Verification items for this drawing (mm, ordinates from the low corner). Coordinates: 2 decimals unless noted, no trailing zeros. Order: outer loops, then holes, each group sorted by start corner. A loop starts at its lowest first (then second) coordinate and runs counter-clockwise, first axis right, second up. Notation, with made-up numbers: (-27, -35.5) -> (-7, -35.5) arc R11 ccw to (-7, -21.5) -> close; hole circle Ø8 at (85, 39.5). An arc over 180 degrees is marked (long way). Answer in a Markdown table with one row per item. Add a question column.
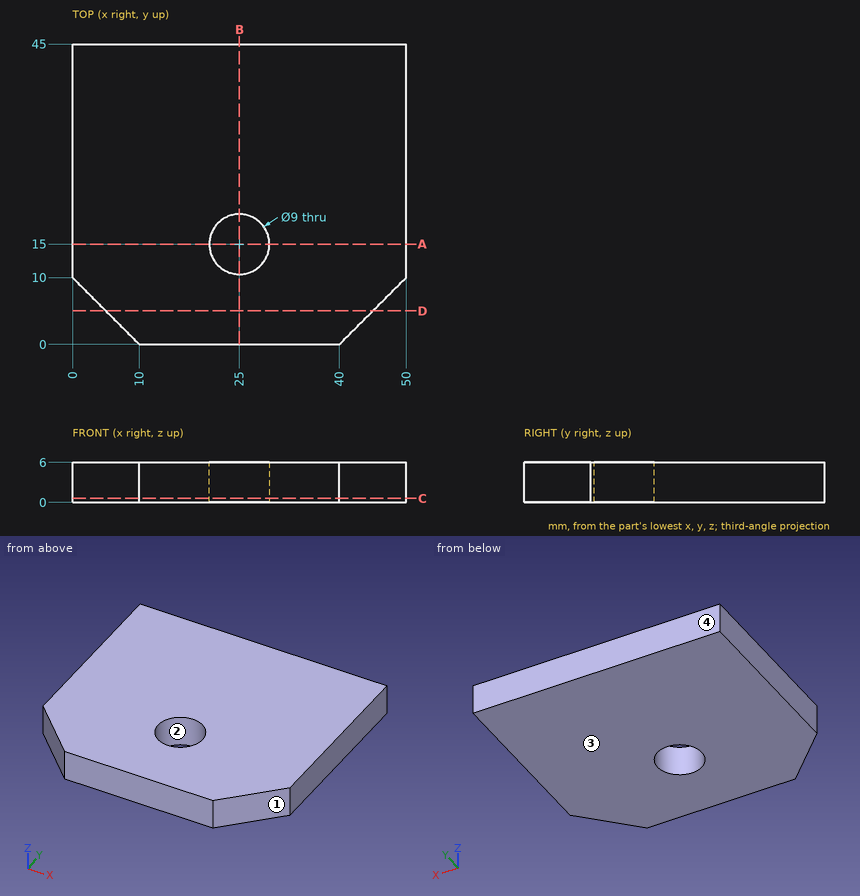
(1) Scan lines: line 1 along Y through (x, z) = (25, 4.15); line 2 along Y through (x, z) = (29, 2.25); line 3 along Y through (x, z) = (46, 0.75). Record each from-to range of solid material in increasing order.
(2) Mould release check, pull along Y, two halves, no side actions. Record for the marked faces 1, 2, 3 and 4: +Y half, -Y half, draft (parallel to the pull), parting line (faces both ways), or undercut.
(3) Cross-section at B-B (x = 25). Enter the section's corners in (y, z).
(4) Cross-section at A-A (y = 15). Enter the section's corners in (x, z).
(5) Cross-section at D-D (y = 5). Enter the section's corners in (x, z), plus the area to 3 significant figures.
(6) Go/stop test with flat-tipped pins: P1, Ø3, axis at x = 7, y = 36, coming from the -Z side; P2, Ø1.5, axis at y = 8.5, z = 2, coming from the -X side; P3, Ø1.5, axis at x = 7, z = 4, coming from the -Y side. Record where each tip stops, or that it passes through.
(7) Cross-section at C-C (z = 0.6). Enter the section's corners in (x, y), plus the area to 3 significant figures.
Checks:
| question | item | result |
|---|---|---|
| 1 | line 1 | 0 to 10.5, 19.5 to 45 |
| 1 | line 2 | 0 to 12.94, 17.06 to 45 |
| 1 | line 3 | 6 to 45 |
| 2 | face 1 | -Y half |
| 2 | face 2 | undercut |
| 2 | face 3 | draft |
| 2 | face 4 | +Y half |
| 3 | outline | (0, 0) -> (10.5, 0) -> (10.5, 6) -> (0, 6) -> close; (19.5, 0) -> (45, 0) -> (45, 6) -> (19.5, 6) -> close |
| 4 | outline | (0, 0) -> (20.5, 0) -> (20.5, 6) -> (0, 6) -> close; (29.5, 0) -> (50, 0) -> (50, 6) -> (29.5, 6) -> close |
| 5 | outline | (5, 0) -> (45, 0) -> (45, 6) -> (5, 6) -> close |
| 5 | area | 240 mm² |
| 6 | P1 | z = 0 |
| 6 | P2 | x = 0.75 |
| 6 | P3 | y = 2.25 |
| 7 | outline | (0, 10) -> (10, 0) -> (40, 0) -> (50, 10) -> (50, 45) -> (0, 45) -> close; hole circle Ø9 at (25, 15) |
| 7 | area | 2,090 mm² |
